```python
from build123d import *

# Parameters (mm, degrees)
SKETCH1_W      = 18
SKETCH1_H      = 18
BASEHEAD_DEPTH = 8
SKETCH2_R      = 6
BASEBODY_DEPTH = 110


with BuildPart() as part:
    # Sketch1 → BaseHead (new body)
    with BuildSketch(Plane(origin=(0, 0, 0), x_dir=(0, 0, -1), z_dir=(1, 0, 0))):
        Rectangle(SKETCH1_W, SKETCH1_H)
    extrude(amount=BASEHEAD_DEPTH)

    # Sketch4 → HeadChamfer (revolve, cut)
    with BuildSketch(Plane(origin=(-7.181436497, -8, 8), x_dir=(-1, 0, 0), z_dir=(0, -0.7071067811865485, -0.7071067811865466))):
        Polygon((-7.181436497, 20.313708499), (-7.181436497, 24.04163056), (-8.538289163, 24.04163056), align=None)
    revolve(axis=Axis((8.946843605, 0, 0), (-1, 0, 0)), mode=Mode.SUBTRACT)

    # Sketch2 → BaseBody (add)
    with BuildSketch(Plane(origin=(8, 0, 0), x_dir=(0, 0, -1), z_dir=(1, 0, 0))):
        Circle(SKETCH2_R)
    extrude(amount=BASEBODY_DEPTH)

    # Sketch5 → Cut-Revolve1 (revolve, cut)
    with BuildSketch(Plane(origin=(-43.209051362, 5, 0), x_dir=(-1, 0, 0), z_dir=(0, 0, 1))):
        Polygon((-131.209051362, 11), (-51.209051362, 11), (-51.209051362, 10.053), (-126.909051362, 10.053), align=None)
    revolve(axis=Axis((-3.790948638, 0, 0), (1, 0, 0)), mode=Mode.SUBTRACT)


solid = part.part
```
Verification items for the finished model (mm, model axes). A direction names the side the tool comes from. Coordinates: 2 decimals unless noted, no trailing zeros. Write each loop counter-clockwise with the first axis right and the second up, starting at its lowest first coordinate (ties: lowest second). Pieces come first, ordered by that corner, then holes. Notation, with made-up numbers: M 29.25,-16 L 55.25,-16 A28 ccw 55.25,19 Z; hole C -21.75,19 d11. An arc over 180 degrees is marked long. One line per item, written item: value.
Item 1: Scan lines: line 1 along Y through (x, z) = (80, 0.25); line 2 along X through (y, z) = (6.75, 4). Record each from-to range of solid material in increasing order.
Check sheet entries:
line 1: y = -5.05 to 5.05
line 2: x = 0 to 8
Item 2: Section check A-A, the plane x = 102. Record the boundary of the cut face in (y, z), plus the area to 3 significant figures.
Check sheet entries:
outline: C 0,0 d12
area: 113 mm^2
Item 3: Gauge pin test, flat ends, axial feed: pin 1 Ø5 at (x, z) = (101, 1) entering from +Y; pin 2 Ø4 at (x, z) = (80, 0) entering from -Y; pin 3 Ø1 at (x, y) = (49, 0) entering from -Z. Record the tip position at first contact, or that the pin passes through.
Check sheet entries:
pin 1: stops at y = 6
pin 2: stops at y = -5.05
pin 3: stops at z = -5.05
Item 4: Access from +Z, -Z, +X, -X, +Y, -Y to the whole of each face (thin tool, end or side, straight path). Record for faces 4 (the flat face through (118, 0, 0)), 5 (the cylindrical face through (46.38, 5.05, -0.22)), 6 (the cylindrical face through (102.79, 1.802, -5.723)).
Check sheet entries:
face 4: +Z, -Z, +X, +Y, -Y
face 5: none
face 6: +X
Item 5: Section check B-B, the plane x = 40. Record the boundary of the cut face in (y, z), plus the area to 3 significant figures.
Check sheet entries:
outline: C 0,0 d10.11
area: 80.2 mm^2
Item 6: Mould release check, pull along X, two halves, no side actions. Record for faces 1 (the conical face through (0.323, 6.967, 7.018)), 2 (the conical face through (84.92, 4.22, 3.24)), 3 (the flat face through (4, -9, 0)): pulls with the +X half, pulls with the -X half, needs draft (parallel to the pull), parting line crosses it, or undercut.
Check sheet entries:
face 1: pulls with the -X half
face 2: undercut
face 3: needs draft
